Can you work these out from the drawing? Everything is in mm from the part's minimum corner. Coordinates: 2 decimals unless noted, no trailing zeros. Order: outer loops, then holes, each group sorted by start corner. A loop starts at its lowest first (then second) coordinate and runs counter-clockwise, first axis right, second up. Notation, with made-up numbers: (-38, 3) -> (-32, 3) arc R25 cw to (-32, 22) -> close; hole circle Ø5 at (-23, 36.5). An arc over 180 degrees is marked (long way). Return JSON: item names as keys, results as strings. Group by question number.
1) If I drill on probe 1 along Y at (x, z) = (4, 15); probe 2 along Z at (x, y) = (0.75, 18); probe 3 along Z at (x, y) = (0.5, 10.5), over which ranges is the centre line in solid material (lowest first)? Write a range as from..to.
2) Thinking about a two-plate mould opening in Y: for the marked faces 1, 2 and 3, which applies, +Y half, -Y half, draft (parallel to the pull), parting line (faces both ways), or undercut?
3) If we section it at A-A, the plane y = 15: Please give me the cut outline in (x, z), then the cut area to 3 significant figures.
4) If we section it at D-D, the plane x = 6.25: Please give me the cut outline in (y, z).
5) If we section it at C-C, the plane x = 2.5: Please give me the cut outline in (y, z).
6) For pin 1 (1 mm diameter, centred on x = 3.5, y = 12.5, fed in from +Z); pin 2 (4 mm diameter, centred on x = 3.5, z = 11.5, fed in from -Y); pin 3 (1 mm diameter, centred on x = 3.5, z = 25.5, fed in from -Y), each with a flat end and sliding along its axis, tell me the tip position at first contact or that it passes through.
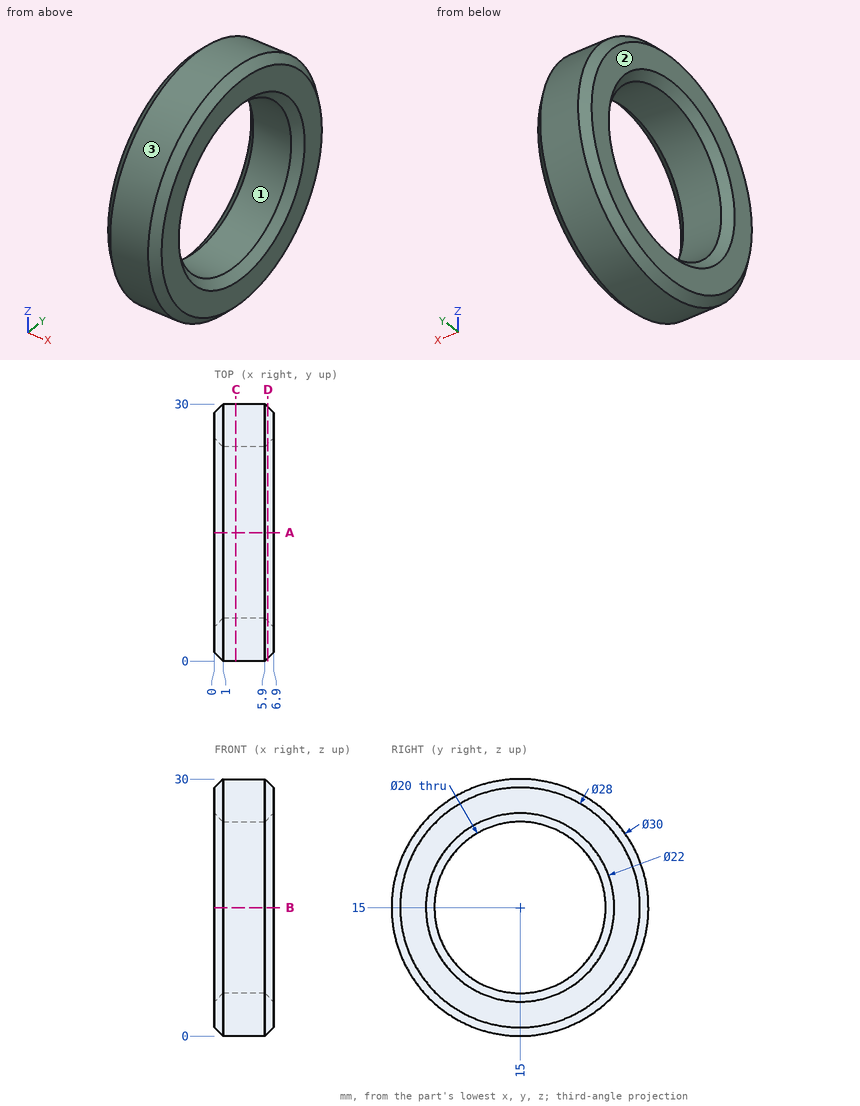
Result sheet:
{
 "1": {"probe 1": "y = 0..5, 25..30", "probe 2": "z = 0.56..5.2, 24.8..29.44", "probe 3": "z = 1.22..5.51, 24.49..28.78"},
 "2": {"face 1": "undercut", "face 2": "draft", "face 3": "parting line"},
 "3": {"outline": "(0, 1) -> (1, 0) -> (5.9, 0) -> (6.9, 1) -> (6.9, 4) -> (5.9, 5) -> (1, 5) -> (0, 4) -> close; (0, 26) -> (1, 25) -> (5.9, 25) -> (6.9, 26) -> (6.9, 29) -> (5.9, 30) -> (1, 30) -> (0, 29) -> close", "area": "65.0 mm2"},
 "4": {"outline": "circle Ø29.3 at (15, 15); hole circle Ø20.7 at (15, 15)"},
 "5": {"outline": "circle Ø30 at (15, 15); hole circle Ø20 at (15, 15)"},
 "6": {"pin 1": "stops at z = 29.87", "pin 2": "stops at y = 0.08", "pin 3": "stops at y = 3.82"}
}
